from build123d import *

# Parameters (mm, degrees)
EXTRUDE_1_DEPTH = 95


with BuildPart() as part:
    # 草图2 → 拉伸-薄壁1 (new, symmetric)
    with BuildSketch(Plane.XY):
        with BuildLine():
            Line((22.25, 540), (22.25, 0))
            ThreePointArc((22.25, 0), (0, -22.25), (-22.25, 0))
            Line((-22.25, 0), (-22.25, 540))
            ThreePointArc((-22.25, 540), (0, 562.25), (22.25, 540))
        make_face()
        with BuildLine():
            Line((20.25, 540), (20.25, 0))
            ThreePointArc((20.25, 0), (0, -20.25), (-20.25, 0))
            Line((-20.25, 0), (-20.25, 540))
            ThreePointArc((-20.25, 540), (0, 560.25), (20.25, 540))
        make_face(mode=Mode.SUBTRACT)
    extrude(amount=EXTRUDE_1_DEPTH, both=True)


solid = part.part
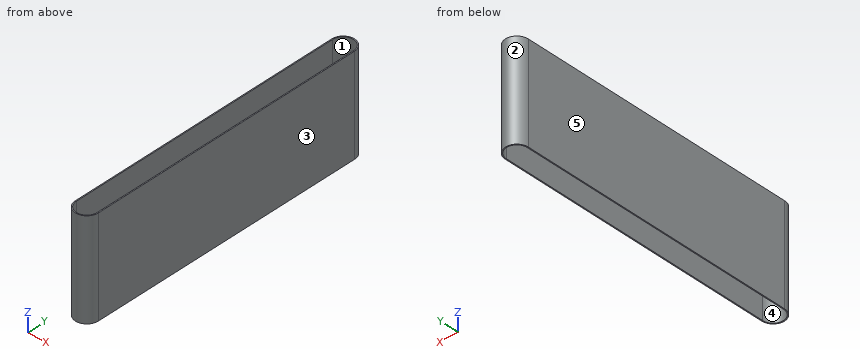
Design review of the part built by this model. Coordinates are the model's own, in mm. Face numbers are marked on the shaded views. A direction names the side the tool comes from. Coordinates: 2 decimals unless noted, no trailing zeros. Order: outer loops, then holes, each group sorted by start corner. A loop starts at its lowest first (then second) coordinate and runs counter-clockwise, first axis right, second up. Notation, with made-up numbers: M -16.75,62.5 L 13.25,62.5 A35 cw 13.25,95.5 Z; hole C -7.75,12.25 d5. An arc over 180 degrees is marked long. Use a Markdown table: item, result.
(1) Add section C-C (x = -13). Give the boundary of the cut face in (y, z).
Worked answers:
| item | result |
|---|---|
| outline | M -18.06,-95 L -15.53,-95 L -15.53,95 L -18.06,95 Z; M 555.53,-95 L 558.06,-95 L 558.06,95 L 555.53,95 Z |
(2) For P1, Ø8, axis at x = -16, z = 71, coming from the -Y side; P2, Ø1, axis at x = -3, z = -51.5, coming from the -Y side; P3, Ø1, axis at x = -7.5, z = -71, coming from the +Y side, all flat-tipped, find the tip position at first contact; note any pin that passes through.
Worked answers:
| item | result |
|---|---|
| P1 | stops at y = -18.74 |
| P2 | stops at y = -22.11 |
| P3 | stops at y = 561.12 |
(3) Draft analysis for pull direction Y (two halves, no side actions). For the marked faces 1, 2 and 3, state which applies: released by +Y, released by -Y, zero draft, split by the parting line, or undercut.
Worked answers:
| item | result |
|---|---|
| face 1 | undercut |
| face 2 | released by +Y |
| face 3 | zero draft |
(4) Wall thickness on probe 1 along X at (y, z) = (455, 11); probe 2 along Y at (x, z) = (11, -12); probe 3 along Y at (x, z) = (12, 63): over which ranges is each line inside the solid? List them lowest first.
Worked answers:
| item | result |
|---|---|
| probe 1 | x = -22.25 to -20.25, 20.25 to 22.25 |
| probe 2 | y = -19.34 to -17, 557 to 559.34 |
| probe 3 | y = -18.74 to -16.31, 556.31 to 558.74 |
(5) Add section A-A (y = 468.5). Give the boundary of the cut face in (x, z).
Worked answers:
| item | result |
|---|---|
| outline | M -22.25,-95 L -20.25,-95 L -20.25,95 L -22.25,95 Z; M 20.25,-95 L 22.25,-95 L 22.25,95 L 20.25,95 Z |
(6) For the marked faces 4 and 5, list the 3-axis set-ups (+Z, -Z, +X, -X, +Y, -Y) from which the entire face can be reached by the end or side of a thin tool; tool diameter is ignored.
Worked answers:
| item | result |
|---|---|
| face 4 | +Z, -Z |
| face 5 | +Z, -Z, -X, +Y, -Y |
(7) Add section B-B (z = 51). Give the boundary of the cut face in (x, y), then the cut area to 3 significant figures.
Worked answers:
| item | result |
|---|---|
| outline | M -22.25,0 A22.25 ccw 22.25,0 L 22.25,540 A22.25 ccw -22.25,540 Z; hole M -20.25,0 A20.25 ccw 20.25,0 L 20.25,540 A20.25 ccw -20.25,540 Z |
| area | 2,430 mm2 |
